CAD build for the part. Positions are in the model's coordinates, mm. A direction names the side the tool comes from. Round coordinates to 2 decimals unless told otherwise and drop trailing zeros. Write each loop counter-clockwise with the first axis right and the second up, starting at its lowest first coordinate (ties: lowest second). Pieces come first, ordered by that corner, then holes. Notation, with made-up numbers: (5, 55) - (23, 55) arc R32 ccw to (23, 92) - close; hole circle Ø7 at (9, -25). An arc over 180 degrees is marked (long way). Use one line per item in the form item = value. Start each with the question number.
Item 1: Drill centre lines: L1, parallel to Y at x = 3.5, z = -2.5; L2, parallel to Y at x = -4.25, z = -4.75; L3, parallel to X at y = 61, z = -2.5. Where is each one in solid material? Low to high.
Item 2: Band-saw the part on B-B, the plane y = 23. List the corners of the cut face in (x, z).
Item 3: Pin check, flat tips, straight feed: pin 1 (4 mm diameter, centred on y = 13.5, z = -3, fed in from +X); pin 2 (2 mm diameter, centred on x = -2, z = 5, fed in from -Y); pin 3 (1 mm diameter, centred on x = 2.5, z = 2, fed in from -Y). Stop position of each tip, or through.
Item 4: Tool access for faces 5 (the cylindrical face through (-0.9, 29.83, -2.86)), 6 (the flat face through (3, 67, 1)), 7 (the flat face through (-1.5, 84, 2.6)), 8 (the flat face through (-3, 87, 3)): list every direction of +Z, -Z, +X, -X, +Y, -Y with a clear straight run to the whole face (end or side of a thin tool).
Item 5: Pull direction Z, two halves, no side cores. Call faces 1 (the flat face through (-3, 84, 0)), 2 (the cylindrical face through (-0.9, 71.93, -2.86)), 3 (the flat face through (3, 84, 0)), 4 (the flat face through (3, 77, 1)): +Z half, -Z half, draft (parallel to the pull), parting line (faces both ways), or undercut.
from build123d import *

# Parameters (mm, degrees)
SKETCH1_R           = 3
BOSS_EXTRUDE1_DEPTH = 45
SKETCH2_R           = 3
BOSS_EXTRUDE2_DEPTH = 15
SKETCH3_R           = 6.5
BOSS_EXTRUDE3_DEPTH = 7
SKETCH4_R           = 3
BOSS_EXTRUDE4_DEPTH = 10
SKETCH5_R           = 6.5
BOSS_EXTRUDE5_DEPTH = 10
CUT_EXTRUDE1_DEPTH  = 6
CHAMFER1_SIZE       = 0.5


with BuildPart() as part:
    # Sketch1 → Boss-Extrude1 (new body)
    with BuildSketch(Plane(origin=(0, 0, 0), x_dir=(1, 0, 0), z_dir=(0, 1, 0))):
        with Locations(Location((0, 0, 0), (0, 0, 90))):
            Circle(SKETCH1_R)
    extrude(amount=BOSS_EXTRUDE1_DEPTH)

    # Sketch2 → Boss-Extrude2 (add)
    with BuildSketch(Plane(origin=(0, 45, 0), x_dir=(1, 0, 0), z_dir=(0, 1, 0))):
        with Locations(Location((0, 0, 0), (0, 0, 90))):
            Circle(SKETCH2_R)
    extrude(amount=BOSS_EXTRUDE2_DEPTH)

    # Sketch3 → Boss-Extrude3 (add)
    with BuildSketch(Plane(origin=(0, 60, 0), x_dir=(1, 0, 0), z_dir=(0, 1, 0))):
        with Locations(Location((0, 0, 0), (0, 0, 270))):
            Circle(SKETCH3_R)
    extrude(amount=BOSS_EXTRUDE3_DEPTH)

    # Sketch4 → Boss-Extrude4 (add)
    with BuildSketch(Plane(origin=(0, 67, 0), x_dir=(1, 0, 0), z_dir=(0, 1, 0))):
        with Locations(Location((0, 0, 0), (0, 0, 90))):
            Circle(SKETCH4_R)
    extrude(amount=BOSS_EXTRUDE4_DEPTH)

    # Sketch5 → Boss-Extrude5 (add)
    with BuildSketch(Plane(origin=(0, 77, 0), x_dir=(1, 0, 0), z_dir=(0, 1, 0))):
        with Locations(Location((0, 0, 0), (0, 0, 270))):
            Circle(SKETCH5_R)
    extrude(amount=BOSS_EXTRUDE5_DEPTH)

    # Sketch6 → Cut-Extrude1 (cut)
    with BuildSketch(Plane(origin=(0, 87, 0), x_dir=(1, 0, 0), z_dir=(0, 1, 0))):
        Polygon((0, 3.464101615), (-3, 1.732050808), (-3, -1.732050808), (0, -3.464101615), (3, -1.732050808), (3, 1.732050808), align=None)
    extrude(amount=-CUT_EXTRUDE1_DEPTH, mode=Mode.SUBTRACT)

    # Chamfer1
    chamfer1_edges = [part.edges().sort_by_distance(p)[0] for p in [
        (0, 77, -6.5),
        (0, 87, -6.5),
        (0, 0, 3),
        (0, 60, -6.5),
        (0, 67, -6.5),
    ]]
    chamfer(chamfer1_edges, length=CHAMFER1_SIZE)


solid = part.part
Determined:
q1.L1 = 60 to 67, 77 to 87
q1.L2 = 60.37 to 66.63, 77.37 to 86.63
q1.L3 = -6 to 6
q2.outline = circle Ø6 at (0, 0)
q3.pin_1 = 2.83
q3.pin_2 = 60
q3.pin_3 = 0.2
q4.face_5 = -Y
q4.face_6 = none
q4.face_7 = +Y
q4.face_8 = +Z, -Z, +X, -X, +Y
q5.face_1 = undercut
q5.face_2 = parting line
q5.face_3 = undercut
q5.face_4 = draft
